Work out the finished part from the listing and answer in its coordinate system (mm). A direction names the side the tool comes from. Coordinates: 2 decimals unless noted, no trailing zeros. Loops run counter-clockwise (first coordinate to the right, second up) from the corner with the lowest first, then second, coordinate; pieces in that order, holes last. Notation, with made-up numbers: (41.5, 28.25) - (79.5, 28.25) arc R17 ccw to (79.5, 49.25) - close; hole circle Ø4 at (21, 42.25). An arc over 180 degrees is marked (long way). Write each question's results on one line, items separated by ' | '. Start each with the question number.
Item 1: Section A-A, the plane x = 0 is taken. Write down the section's boundary in (y, z), plus the area to 3 significant figures.
Item 2: For a pull along Z with two mould halves and no side action, classify faces 1 (the face through (-52, 12, 53)), 2 (the face through (-29, 7, -29)), 3 (the face through (-1, 12, -55)) as +Z half, -Z half, draft (parallel to the pull), parting line (faces both ways), or undercut.
Item 3: Each of these flat-tipped pins is pushed along its axis until it touches: pin 1 Ø4 at (x, z) = (35.5, 24.5) entering from -Y; pin 2 Ø5.5 at (x, z) = (32.5, 32.5) entering from -Y; pin 3 Ø4 at (x, z) = (-14.5, 27.5) entering from +Y; pin 4 Ø4.5 at (x, z) = (32, -29.5) entering from +Y. Where does it stop, or does it pass through?
Item 4: A tool of negligible diameter and unlimited length cuts with its end or side. For faces 4 (the face through (36, 7, -29)), 5 (the face through (-25, -2, -14)), from which of +Z, -Z, +X, -X, +Y, -Y can it reach the whole face along a straight path? Write none if from no direction.
Item 5: Consider probe 1 along Z at (x, y) = (32.5, 12); probe 2 along Z at (x, y) = (-44.45, 14.5); probe 3 along X at (y, z) = (2.25, 32.5). Determine where each line is inside the solid, lowest interval first. Write a range as [from, to].
Item 6: Section B-B, the plane y = 17 is taken. Count the separate pieces of the cut face and the enclosed holes in it, plus the area to 3 significant figures.
from build123d import *

# Parameters (mm, degrees)
SKETCH_1_W                     = 110
SKETCH_1_H                     = 110
EXTRUDE_1_DEPTH                = 25
SKETCH_3_R                     = 31.25
SKETCH_3_R_2                   = 28.25
EXTRUDE_2_DEPTH                = 2
SKETCH_4_R                     = 28.25
CUT_EXTRUDE_1_DEPTH            = 82.700673192
SKETCH_5_R                     = 42.5
CUT_EXTRUDE_2_DEPTH            = 6.5
HOLE_WIZARD_M8_1_D             = 6.8
HOLE_WIZARD_M8_1_DEPTH         = 19.75
HOLE_WIZARD_M8_1_TIP           = 2.042926105
HOLE_WIZARD_M8_1_2_D           = 9
HOLE_WIZARD_M8_1_2_CBORE_D     = 15
HOLE_WIZARD_M8_1_2_CBORE_DEPTH = 18
CHAMFER_1_SIZE                 = 5
CHAMFER_2_SIZE                 = 1
CHAMFER_3_SIZE                 = 0.5


with BuildPart() as part:
    # 草图1 → 凸台-拉伸1 (new body)
    with BuildSketch(Plane(origin=(0, 0, 0), x_dir=(1, 0, 0), z_dir=(0, 1, 0))):
        Rectangle(SKETCH_1_W, SKETCH_1_H)
    extrude(amount=EXTRUDE_1_DEPTH)

    # 草图3 → 凸台-拉伸2 (add)
    with BuildSketch(Plane.XZ):
        with Locations(Location((0, 0, 0), (0, 0, 270))):
            Circle(SKETCH_3_R)
        with Locations(Location((0, 0, 0), (0, 0, 270))):
            Circle(SKETCH_3_R_2, mode=Mode.SUBTRACT)
    extrude(amount=EXTRUDE_2_DEPTH)

    # 草图4 → 切除-拉伸1 (cut, through all)
    with BuildSketch(Plane.XZ):
        with Locations(Location((0, 0, 0), (0, 0, 270))):
            Circle(SKETCH_4_R)
    extrude(amount=-CUT_EXTRUDE_1_DEPTH, mode=Mode.SUBTRACT)

    # 草图5 → 切除-拉伸2 (cut)
    with BuildSketch(Plane(origin=(0, 25, 0), x_dir=(1, 0, 0), z_dir=(0, 1, 0))):
        with Locations(Location((0, 0, 0), (0, 0, 270))):
            Circle(SKETCH_5_R)
    extrude(amount=-CUT_EXTRUDE_2_DEPTH, mode=Mode.SUBTRACT)

    # Hole Wizard M8 _1
    with Locations(Plane(origin=(0, 25, 0), x_dir=(1, 0, 0), z_dir=(0, 1, 0))):
        with Locations((-44.45, 44.45), (0, 0), (44.45, 44.45), (-44.45, -44.45), (44.45, -44.45)):
            Hole(HOLE_WIZARD_M8_1_D / 2, depth=HOLE_WIZARD_M8_1_DEPTH)
            with Locations((0, 0, -(HOLE_WIZARD_M8_1_DEPTH + HOLE_WIZARD_M8_1_TIP / 2))):  # 118° drill point
                Cone(0, HOLE_WIZARD_M8_1_D / 2, HOLE_WIZARD_M8_1_TIP, mode=Mode.SUBTRACT)

    # Hole Wizard M8 _1 2 (through all)
    with Locations(Plane(origin=(0, 25, 0), x_dir=(1, 0, 0), z_dir=(0, 1, 0))):
        with Locations((-32.5, 32.5), (0, 0), (32.5, 32.5), (-32.5, -32.5), (32.5, -32.5)):
            CounterBoreHole(HOLE_WIZARD_M8_1_2_D / 2, HOLE_WIZARD_M8_1_2_CBORE_D / 2, HOLE_WIZARD_M8_1_2_CBORE_DEPTH)

    # 倒角1
    chamfer_1_edges = [part.edges().sort_by_distance(p)[0] for p in [
        (55, 12.5, 55),
        (-55, 12.5, 55),
        (-55, 12.5, -55),
        (55, 12.5, -55),
    ]]
    chamfer(chamfer_1_edges, length=CHAMFER_1_SIZE)

    # 倒角2
    chamfer_2_edges = [part.edges().sort_by_distance(p)[0] for p in [
        (-42.5, 25, 0),
        (42.5, 25, 0),
        (0, 25, 42.5),
        (0, 25, -42.5),
    ]]
    chamfer(chamfer_2_edges, length=CHAMFER_2_SIZE)

    # 倒角3
    chamfer_3_edges = [part.edges().sort_by_distance(p)[0] for p in [
        (0, -2, 31.25),
    ]]
    chamfer(chamfer_3_edges, length=CHAMFER_3_SIZE)


solid = part.part
Answer key:
1) outline: (-2, -30.75) - (-1.5, -31.25) - (0, -31.25) - (0, -55) - (25, -55) - (25, -43.5) - (24, -42.5) - (18.5, -42.5) - (18.5, -28.25) - (-2, -28.25) - close; (-2, 28.25) - (18.5, 28.25) - (18.5, 42.5) - (24, 42.5) - (25, 43.5) - (25, 55) - (0, 55) - (0, 31.25) - (-1.5, 31.25) - (-2, 30.75) - close | area: 1,160 mm^2
2) face 1: +Z half | face 2: undercut | face 3: -Z half
3) pin 1: stops at y = 0 | pin 2: passes through | pin 3: stops at y = 18.5 | pin 4: stops at y = 7
4) face 4: +Y | face 5: +Z, -Z, +X, -X, -Y
5) probe 1: z = [-55, -40], [-25, 25], [40, 55] | probe 2: z = [-55, -47.85], [-41.05, 41.05], [47.85, 55] | probe 3: x = [-55, -37], [-28, 28], [37, 55]
6) separate pieces: 1 | enclosed holes: 9 | area: 8,690 mm^2
